from build123d import *

# Parameters (mm, degrees)
SKETCH_1_R      = 2.5
SKETCH_1_R_2    = 6.25
EXTRUDE_1_DEPTH = 4


with BuildPart() as part:
    # 草图1 → 凸台-拉伸1 (new body)
    with BuildSketch(Plane.XY.offset(2)):
        with BuildLine():
            Line((-20, -10), (20, -10))
            ThreePointArc((20, -10), (23.535533906, -8.535533906), (25, -5))
            Line((25, -5), (25, 5))
            ThreePointArc((25, 5), (23.535533906, 8.535533906), (20, 10))
            Line((20, 10), (-20, 10))
            ThreePointArc((-20, 10), (-23.535533906, 8.535533906), (-25, 5))
            Line((-25, 5), (-25, -5))
            ThreePointArc((-25, -5), (-23.535533906, -8.535533906), (-20, -10))
        make_face()
        with Locations(Location((-17.5, 6, 0), (0, 0, 180))):
            Circle(SKETCH_1_R, mode=Mode.SUBTRACT)
        with Locations(Location((17.5, -6, 0), (0, 0, 180))):
            Circle(SKETCH_1_R, mode=Mode.SUBTRACT)
        with Locations(Location((0, 0, 0), (0, 0, 180))):
            Circle(SKETCH_1_R_2, mode=Mode.SUBTRACT)
    extrude(amount=-EXTRUDE_1_DEPTH)


solid = part.part
Input: part model. Units: mm. Frame: model coordinates. Give positions to 0.01 mm unless a question says otherwise; leave off trailing zeros. Loops run counter-clockwise (first coordinate to the right, second up) from the corner with the lowest first, then second, coordinate; pieces in that order, holes last. Notation, with made-up numbers: M -36.75,30 L -20.75,30 A32 cw -20.75,63 Z; hole C -13,42.25 d1. An arc over 180 degrees is marked long. Use CSV: the item, a comma, the result in double quotes.
(1) Section A-A, the plane y = 0. Return loops of the section in (x, z).
Outcome:
outline,"M -25,-2 L -6.25,-2 L -6.25,2 L -25,2 Z; M 6.25,-2 L 25,-2 L 25,2 L 6.25,2 Z"
(2) Pin query (flat end, axial travel): P1, Ø10, axis at x = 0, y = 0, coming from the -Z side. Return the tip coordinate at first contact, or that it passes through.
Outcome:
P1,"passes through"
(3) Material intervals for L1, parallel to Y at x = 17.5, z = 0.7; L2, parallel to Y at x = 0, z = -0.8; L3, parallel to X at y = -8.25, z = 1.35, sorted ascending. Write a range as [from, to].
Outcome:
L1,"y = [-10, -8.5], [-3.5, 10]"
L2,"y = [-10, -6.25], [6.25, 10]"
L3,"x = [-23.8, 16.41], [18.59, 23.8]"
(4) Pull-direction query (X, two-part tool) for faces 1 (the face through (0, 7, -2)), 2 (the face through (-15, 6, 0)), 3 (the face through (25, 0, 0)), 4 (the face through (-24, -8, 0)); classes: pulls with the +X half, pulls with the -X half, needs draft (parallel to the pull), parting line crosses it, or undercut.
Outcome:
face 1,"needs draft"
face 2,"undercut"
face 3,"pulls with the +X half"
face 4,"pulls with the -X half"
(5) Section C-C, the plane z = -0.6. Return loops of the section in (x, y), plus the area to 3 significant figures.
Outcome:
outline,"M -25,-5 A5 ccw -20,-10 L 20,-10 A5 ccw 25,-5 L 25,5 A5 ccw 20,10 L -20,10 A5 ccw -25,5 Z; hole C -17.5,6 d5; hole C 0,0 d12.5; hole C 17.5,-6 d5"
area,"817 mm²"
(6) Section B-B, the plane x = 17.5. Return loops of the section in (y, z), plus the area to 3 significant figures.
Outcome:
outline,"M -10,-2 L -8.5,-2 L -8.5,2 L -10,2 Z; M -3.5,-2 L 10,-2 L 10,2 L -3.5,2 Z"
area,"60.0 mm²"
